For this review, take the finished solid that the model builds, in its own axes (mm). Round coordinates to 2 decimals unless told otherwise and drop trailing zeros. Order: outer loops, then holes, each group sorted by start corner. A loop starts at its lowest first (then second) coordinate and runs counter-clockwise, first axis right, second up. Notation, with made-up numbers: (-25.75, 15) -> (-15.75, 15) arc R25 cw to (-15.75, 43) -> close; hole circle Ø5 at (-32, -0.5). An arc over 180 degrees is marked (long way). Put each result on its own line as item: value. Start each with the question number.
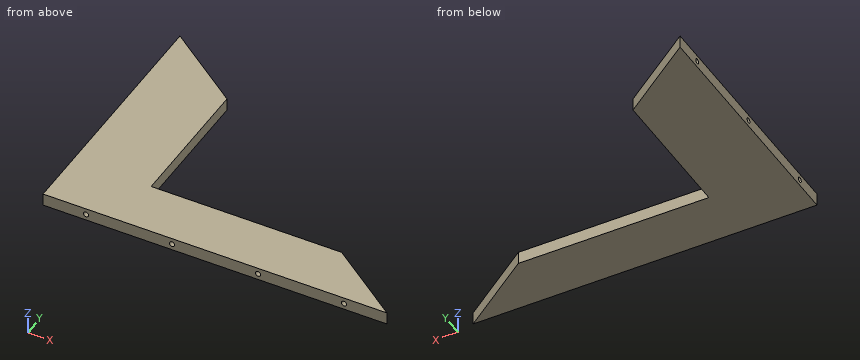
```python
from build123d import *

# Parameters (mm, degrees)
EXTRUDE_1_DEPTH        = 8
HOLE_WIZARD_M4_1_D     = 3.3
HOLE_WIZARD_M4_1_DEPTH = 15
HOLE_WIZARD_M4_1_TIP   = 0.991420021
HOLE_WIZARD_M4_2_D     = 3.3
HOLE_WIZARD_M4_2_DEPTH = 15.1
HOLE_WIZARD_M4_2_TIP   = 0.991420021


with BuildPart() as part:
    # 草图1 → 凸台-拉伸1 (new body)
    with BuildSketch(Plane.XY):
        Polygon((-140, 40), (-140, -120), (80, -120), (31.875, -85), (-90, -85), (-90, 3.636363636), align=None)
    extrude(amount=EXTRUDE_1_DEPTH)

    # M4 螺纹孔1
    with Locations(Plane(origin=(0, -120, 0), x_dir=(-1, 0, 0), z_dir=(0, -1, 0))):
        with Locations((112.5, -4), (57.5, -4), (2.5, -4), (-52.5, -4)):
            Hole(HOLE_WIZARD_M4_1_D / 2, depth=HOLE_WIZARD_M4_1_DEPTH)
            with Locations((0, 0, -(HOLE_WIZARD_M4_1_DEPTH + HOLE_WIZARD_M4_1_TIP / 2))):  # 118° drill point
                Cone(0, HOLE_WIZARD_M4_1_D / 2, HOLE_WIZARD_M4_1_TIP, mode=Mode.SUBTRACT)

    # M4 螺纹孔2
    with Locations(Plane.ZY.offset(140)):
        with Locations((4, 20), (4, -40), (4, -100)):
            Hole(HOLE_WIZARD_M4_2_D / 2, depth=HOLE_WIZARD_M4_2_DEPTH)
            with Locations((0, 0, -(HOLE_WIZARD_M4_2_DEPTH + HOLE_WIZARD_M4_2_TIP / 2))):  # 118° drill point
                Cone(0, HOLE_WIZARD_M4_2_D / 2, HOLE_WIZARD_M4_2_TIP, mode=Mode.SUBTRACT)


solid = part.part
```
Item 1: Consider section B-B, the plane x = -73. Write out the cut boundary in (y, z).
Item 2: Consider section A-A, the plane y = -28.5. Write out the cut boundary in (x, z), plus the area to 3 significant figures.
Item 3: Insertion check: pin 1 Ø2.5 at (x, z) = (-57.5, 4) entering from -Y; pin 2 Ø3 at (x, z) = (52.5, 4) entering from -Y; pin 3 Ø2.5 at (y, z) = (20, 4) entering from +X. Each pin has a flat end and moves straight along its axis. Give the tip position at first contact, or say it passes through.
Item 4: For L1, parallel to Z at x = -134, y = -100; L2, parallel to X at y = -77.5, z = 1; L3, parallel to Y at x = -42, z = 6, list the stretches that pass through material, from the lowest coordinate up.
Evaluation:
1. outline: (-120, 0) -> (-85, 0) -> (-85, 8) -> (-120, 8) -> close
2. outline: (-140, 0) -> (-90, 0) -> (-90, 8) -> (-140, 8) -> close
2. area: 400 mm^2
3. pin 1: stops at y = -104.76
3. pin 2: stops at y = -104.91
3. pin 3: stops at x = -110.78
4. L1: z = 0 to 2.35, 5.65 to 8
4. L2: x = -140 to -90
4. L3: y = -120 to -85
